```python
from build123d import *

# Parameters (mm, degrees)
EXTRUDE_1_DEPTH     = 13.5
EXTRUDE_2_REACH     = 80.583
EXTRUDE_3_DEPTH     = 15
CUT_EXTRUDE_1_DEPTH = 8.5
SKETCH_6_W          = 16
SKETCH_6_H          = 2.5
CUT_EXTRUDE_2_DEPTH = 22
SKETCH_7_R          = 6.5
CUT_EXTRUDE_3_DEPTH = 8
CUT_EXTRUDE_4_REACH = 78.737
SKETCH_8_R          = 4.1


with BuildPart() as part:
    # 草图1 → 凸台-拉伸1 (new, symmetric)
    with BuildSketch(Plane.XY):
        with BuildLine():
            Line((68, 0), (68, 15))
            ThreePointArc((68, 15), (63.909956901, 26.921785896), (55.283946786, 36.111420329))
            ThreePointArc((55.283946786, 36.111420329), (53.929013217, 36.772688008), (52.438560542, 37))
            Line((52.438560542, 37), (-52.438560542, 37))
            ThreePointArc((-52.438560542, 37), (-53.929013217, 36.772688008), (-55.283946786, 36.111420329))
            ThreePointArc((-55.283946786, 36.111420329), (-63.909956901, 26.921785896), (-68, 15))
            Line((-68, 15), (-68, 0))
            Line((-68, 0), (-44, 0))
            Line((-44, 0), (-44, 27))
            ThreePointArc((-44, 27), (-43.121320344, 29.121320344), (-41, 30))
            Line((-41, 30), (41, 30))
            ThreePointArc((41, 30), (43.121320344, 29.121320344), (44, 27))
            Line((44, 27), (44, 0))
            Line((44, 0), (68, 0))
        make_face()
    extrude(amount=EXTRUDE_1_DEPTH, both=True)

    # 凸台-拉伸2: up to this face of the body (flat: up to its plane)
    extrude_2_end = Plane(part.part.faces().sort_by_distance((0, 30, 0))[0])
    # 草图2 → 凸台-拉伸2 (add, up to the picked face)
    with BuildSketch(Plane.XZ, mode=Mode.PRIVATE) as extrude_2_sk1:
        with BuildLine():
            Line((-44, 13.5), (-44, -13.5))
            ThreePointArc((-44, -13.5), (-43, 0), (-44, 13.5))
        make_face()
    extrude_2_tool1 = split(extrude(extrude_2_sk1.sketch, amount=-EXTRUDE_2_REACH, mode=Mode.PRIVATE), bisect_by=extrude_2_end, keep=Keep.BOTH, mode=Mode.PRIVATE)
    # 草图2 → 凸台-拉伸2 (add, up to the picked face)
    with BuildSketch(Plane.XZ, mode=Mode.PRIVATE) as extrude_2_sk2:
        with BuildLine():
            Line((44, 13.5), (44, -13.5))
            ThreePointArc((44, -13.5), (43, 0), (44, 13.5))
        make_face()
    extrude_2_tool2 = split(extrude(extrude_2_sk2.sketch, amount=-EXTRUDE_2_REACH, mode=Mode.PRIVATE), bisect_by=extrude_2_end, keep=Keep.BOTH, mode=Mode.PRIVATE)
    add(extrude_2_tool1.solids().sort_by(Axis((-43.599812, 0, 0), (0, 1, 0)))[0])
    add(extrude_2_tool2.solids().sort_by(Axis((43.599812, 0, 0), (0, 1, 0)))[0])

    # 草图4 → 凸台-拉伸3 (add)
    with BuildSketch(Plane.XZ):
        with BuildLine():
            Line((-68, 13.5), (-68, -13.5))
            ThreePointArc((-68, -13.5), (-69.327123119, 0), (-68, 13.5))
        make_face()
        with BuildLine():
            Line((68, 13.5), (68, -13.5))
            ThreePointArc((68, -13.5), (69.327123119, 0), (68, 13.5))
        make_face()
    extrude(amount=-EXTRUDE_3_DEPTH)

    # 草图5 → 切除-拉伸1 (cut, symmetric)
    with BuildSketch(Plane.XY):
        with BuildLine():
            ThreePointArc((-52.438560542, 37), (-53.929013217, 36.772688008), (-55.283946786, 36.111420329))
            ThreePointArc((-55.283946786, 36.111420329), (-63.909956901, 26.921785896), (-68, 15))
            Line((-68, 15), (-49, 15))
            Line((-49, 15), (-49, 37))
            Line((-49, 37), (-52.438560542, 37))
        make_face()
        with BuildLine():
            ThreePointArc((52.438560542, 37), (53.929013217, 36.772688008), (55.283946786, 36.111420329))
            ThreePointArc((55.283946786, 36.111420329), (63.909956901, 26.921785896), (68, 15))
            Line((68, 15), (49, 15))
            Line((49, 15), (49, 37))
            Line((49, 37), (52.438560542, 37))
        make_face()
    extrude(amount=CUT_EXTRUDE_1_DEPTH, both=True, mode=Mode.SUBTRACT)

    # 草图6 → 切除-拉伸2 (cut)
    with BuildSketch(Plane.XZ):
        with Locations((-55.5, 9.75)):
            Rectangle(SKETCH_6_W, SKETCH_6_H)
        with Locations((55.5, 9.75)):
            Rectangle(SKETCH_6_W, SKETCH_6_H)
        with Locations((55.5, -9.75)):
            Rectangle(SKETCH_6_W, SKETCH_6_H)
        with Locations((-55.5, -9.75)):
            Rectangle(SKETCH_6_W, SKETCH_6_H)
    extrude(amount=-CUT_EXTRUDE_2_DEPTH, mode=Mode.SUBTRACT)

    # 草图7 → 切除-拉伸3 (cut)
    with BuildSketch(Plane(origin=(0, 15, 0), x_dir=(1, 0, 0), z_dir=(0, 1, 0))):
        with Locations(Location((-58.25, 0, 0), (0, 0, 180))):
            Circle(SKETCH_7_R)
        with Locations(Location((58.25, 0, 0), (0, 0, 180))):
            Circle(SKETCH_7_R)
    extrude(amount=-CUT_EXTRUDE_3_DEPTH, mode=Mode.SUBTRACT)

    # 草图8 → 切除-拉伸4 (cut, up to next)
    with BuildSketch(Plane(origin=(0, 7, 0), x_dir=(1, 0, 0), z_dir=(0, 1, 0)), mode=Mode.PRIVATE) as cut_extrude_4_sk1:
        with Locations(Location((58.25, 0, 0), (0, 0, 180))):
            Circle(SKETCH_8_R)
    cut_extrude_4_tool1 = extrude(cut_extrude_4_sk1.sketch, amount=-CUT_EXTRUDE_4_REACH, mode=Mode.PRIVATE) & part.part
    # 草图8 → 切除-拉伸4 (cut, up to next)
    with BuildSketch(Plane(origin=(0, 7, 0), x_dir=(1, 0, 0), z_dir=(0, 1, 0)), mode=Mode.PRIVATE) as cut_extrude_4_sk2:
        with Locations(Location((-58.25, 0, 0), (0, 0, 180))):
            Circle(SKETCH_8_R)
    cut_extrude_4_tool2 = extrude(cut_extrude_4_sk2.sketch, amount=-CUT_EXTRUDE_4_REACH, mode=Mode.PRIVATE) & part.part
    add(cut_extrude_4_tool1.solids().sort_by_distance((58.25, 7, 0))[0], mode=Mode.SUBTRACT)
    add(cut_extrude_4_tool2.solids().sort_by_distance((-58.25, 7, 0))[0], mode=Mode.SUBTRACT)


solid = part.part
```
Check sheet for the modelled part. Datum: model origin and axes. Units: mm. A direction names the side the tool comes from. Coordinates: 2 decimals unless noted, no trailing zeros. Order: outer loops, then holes, each group sorted by start corner. A loop starts at its lowest first (then second) coordinate and runs counter-clockwise, first axis right, second up. Notation, with made-up numbers: M 36,67 L 48,67 A22 ccw 48,75 Z; hole C -16.5,14.25 d10. An arc over 180 degrees is marked long. Write each question's results on one line, items separated by ' | '. Start each with the question number.
1. Mould release check, pull along X, two halves, no side actions. Record for faces 4 (the face through (-1, 30, 0)), 5 (the face through (-69.327, 7.395, -0.19)), 6 (the face through (-56, 8, 8.5)), 7 (the face through (1, 37, 0)): +X half, -X half, draft (parallel to the pull), parting line (faces both ways), or undercut.
2. Cross-section at C-C on x = 58.25. Record the cut outline in (y, z).
3. Material ranges on probe 1 along Z at (x, y) = (-58, 3); probe 2 along Z at (x, y) = (-58.25, 10); probe 3 along Y at (x, z) = (32, -7.25), recorded low to high.
4. Cross-section at A-A on y = 13. Record the cut outline in (x, z) (3 decimals), and give its area (3 significant figures).
5. Cross-section at D-D on y = 24. Record the cut outline in (x, z) (3 decimals).
6. Access from +Z, -Z, +X, -X, +Y, -Y to the whole of each face (thin tool, end or side, straight path). Record for faces 1 (the face through (-62.5, 7, 0.1)), 2 (the face through (47.5, 11, 10)), 3 (the face through (-57, 26, 8.5)).
7. Go/stop test with flat-tipped pins: P1, Ø2, axis at x = -29.5, z = 7, coming from the -Y side; P2, Ø6, axis at x = -61.5, z = 4.5, coming from the +Y side; P3, Ø10.5, axis at x = 58.25, z = 0, coming from the +Y side. Record where each tip stops, or that it passes through.
8. Cross-section at B-B on z = -1.5. State how many separate pieces and enclosed holes the cut face has, and give its area (3 significant figures).
Checks:
1) face 4: undercut | face 5: -X half | face 6: undercut | face 7: draft
2) outline: M 0,-13.5 L 33.77,-13.5 L 33.77,-8.5 L 22,-8.5 L 22,-11 L 0,-11 Z; M 0,-8.5 L 15,-8.5 L 15,-6.5 L 7,-6.5 L 7,-4.1 L 0,-4.1 Z; M 0,4.1 L 7,4.1 L 7,6.5 L 15,6.5 L 15,8.5 L 0,8.5 Z; M 0,11 L 22,11 L 22,8.5 L 33.77,8.5 L 33.77,13.5 L 0,13.5 Z
3) probe 1: z = -13.5 to -11, -8.5 to -4.09, 4.09 to 8.5, 11 to 13.5 | probe 2: z = -13.5 to -11, -8.5 to -6.5, 6.5 to 8.5, 11 to 13.5 | probe 3: y = 30 to 37
4) outline: M -68,-13.5 L -44,-13.5 A91.625 ccw -44,13.5 L -68,13.5 A69.327 ccw Z; M 44,-13.5 L 68,-13.5 A69.327 ccw 68,13.5 L 44,13.5 A91.625 ccw Z; hole C -58.25,0 d13; hole M -63.5,-11 L -47.5,-11 L -47.5,-8.5 L -63.5,-8.5 Z; hole M -63.5,8.5 L -47.5,8.5 L -47.5,11 L -63.5,11 Z; hole M 47.5,-11 L 63.5,-11 L 63.5,-8.5 L 47.5,-8.5 Z; hole M 47.5,8.5 L 63.5,8.5 L 63.5,11 L 47.5,11 Z; hole C 58.25,0 d13 | area: 954 mm²
5) outline: M -65.457,-13.5 L -44,-13.5 A91.625 ccw -44,13.5 L -65.457,13.5 L -65.457,8.5 L -49,8.5 L -49,-8.5 L -65.457,-8.5 Z; M 44,-13.5 L 65.457,-13.5 L 65.457,-8.5 L 49,-8.5 L 49,8.5 L 65.457,8.5 L 65.457,13.5 L 44,13.5 A91.625 ccw Z
6) face 1: +Y | face 2: -Y | face 3: -X, +Y
7) P1: stops at y = 30 | P2: stops at y = 15 | P3: stops at y = 7
8) separate pieces: 3 | enclosed holes: 0 | area: 1,350 mm²
